Could you check a few things on this model? Use its own coordinates, in mm. Round coordinates to 2 decimals unless told otherwise and drop trailing zeros. Write each loop counter-clockwise with the first axis right and the second up, starting at its lowest first coordinate (ties: lowest second). Pieces come first, ordered by that corner, then holes. Notation, with made-up numbers: M 7,-9 L 15,-9 A11 cw 15,-4 Z; hole C 11,-12 d5. An arc over 180 degrees is marked long. One line per question, with ' | ' between items. Start each with the question number.
```python
from build123d import *

# Parameters (mm, degrees)
BOSS_EXTRUDE1_DEPTH = 8
SKETCH2_R           = 6.25
CUT_EXTRUDE1_DEPTH  = 224.546415762


with BuildPart() as part:
    # Sketch1 → Boss-Extrude1 (new body)
    with BuildSketch(Plane(origin=(0, 0, 0), x_dir=(-1, 0, 0), z_dir=(0, 0, 1))):
        with BuildLine():
            Line((-106.85, 12), (-135, 12))
            Line((-135, 12), (-135, -178))
            Line((-135, -178), (135, -178))
            Line((135, -178), (135, 12))
            Line((135, 12), (106.85, 12))
            Line((106.85, 12), (106.85, 0))
            ThreePointArc((106.85, 0), (0, -106.85), (-106.85, 0))
            Line((-106.85, 0), (-106.85, 12))
        make_face()
    extrude(amount=BOSS_EXTRUDE1_DEPTH)

    # Sketch2 → Cut-Extrude1 (cut, through all)
    with BuildSketch(Plane(origin=(0, 0, 0), x_dir=(-1, 0, 0), z_dir=(0, 0, -1))):
        with Locations((-116.913429511, 67.5)):
            Circle(SKETCH2_R)
        with Locations((116.913429511, 67.5)):
            Circle(SKETCH2_R)
        with Locations((0, 135)):
            Circle(SKETCH2_R)
    extrude(amount=-CUT_EXTRUDE1_DEPTH, mode=Mode.SUBTRACT)


solid = part.part
```
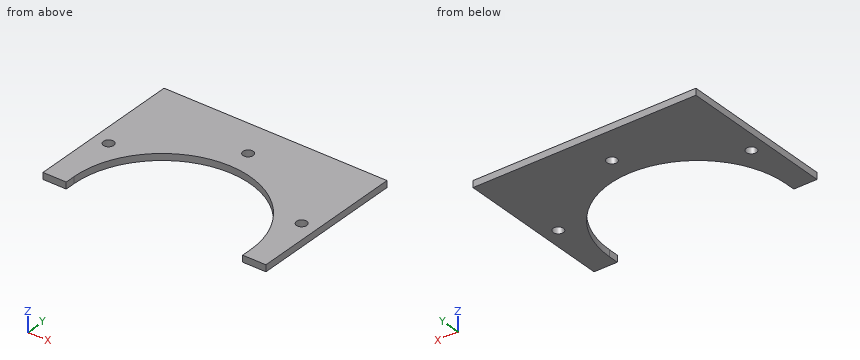
1. I need wall thicknesses on line 1 along Y through (x, z) = (0, 5.75); line 2 along X through (y, z) = (19, 0.75); line 3 along X through (y, z) = (46, 1.75). Which ranges of each line are inside material? Lowest first, please. Write a range as from..to.
2. I'm going to push flat-ended pins straight in: P1, Ø11, axis at x = -116.91, y = 67.5, coming from the +Z side; P2, Ø3, axis at x = 82.5, z = 4, coming from the -Y side. Where does each tip first touch, or does it pass through?
3. Suppose I cut it at C-C (x = 0). Write out the boundary of the cut face in (y, z).
4. Suppose I cut it at A-A (y = 135). Write out the boundary of the cut face in (x, z).
5. Suppose I cut it at D-D (y = 67.5). Write out the boundary of the cut face in (x, z), and give its area (3 significant figures).
6. Suppose I cut it at B-B (z = 2). Write out the boundary of the cut face in (x, y).
Computed:
1) line 1: y = 106.85..128.75, 141.25..178 | line 2: x = -135..-105.15, 105.15..135 | line 3: x = -135..-96.44, 96.44..135
2) P1: passes through | P2: stops at y = 66.04
3) outline: M 106.85,0 L 128.75,0 L 128.75,8 L 106.85,8 Z; M 141.25,0 L 178,0 L 178,8 L 141.25,8 Z
4) outline: M -135,0 L -6.25,0 L -6.25,8 L -135,8 Z; M 6.25,0 L 135,0 L 135,8 L 6.25,8 Z
5) outline: M -135,0 L -123.16,0 L -123.16,8 L -135,8 Z; M -110.66,0 L -82.83,0 L -82.83,8 L -110.66,8 Z; M 82.83,0 L 110.66,0 L 110.66,8 L 82.83,8 Z; M 123.16,0 L 135,0 L 135,8 L 123.16,8 Z | area: 635 mm²
6) outline: M -135,-12 L -106.85,-12 L -106.85,0 A106.85 cw 106.85,0 L 106.85,-12 L 135,-12 L 135,178 L -135,178 Z; hole C -116.91,67.5 d12.5; hole C 0,135 d12.5; hole C 116.91,67.5 d12.5
